Study the drawing (mm; zero at the part's minimum x, y, z) and answer. A direction names the side the tool comes from. Round coordinates to 2 decimals unless told otherwise and drop trailing zeros. Write each loop counter-clockwise with the first axis right and the second up, starting at its lowest first coordinate (ties: lowest second). Pieces come first, ordered by that corner, then holes.
(1) Each of these flat-tipped pins is pushed along its axis until it touches: pin 1 Ø1 at (x, y) = (1.5, 6.5) entering from -Z; pin 2 Ø0.7 at (x, y) = (3, 2) entering from +Z. Where does it stop, or does it pass through?
(2) Find the intervals of material crossed by probe 1 along Z at (x, y) = (2.35, 2.5); probe 2 along X at (y, z) = (3.75, 2.35); probe 3 along X at (y, z) = (22.75, 1.5), in increasing order.
(3) A cutting plane is placed at A-A, the plane y = 21.25. Give the vertices of the cut face in (x, z).
(4) For the marked faces 1 and 2, determine the directions among +Z, -Z, +X, -X, +Y, -Y from which every point of the face is accessible in a straight line to the end or side of a thin tool.
(5) A cutting plane is placed at B-B, the plane y = 3. Give the vertices of the cut face in (x, z), and give its area (3 significant figures).
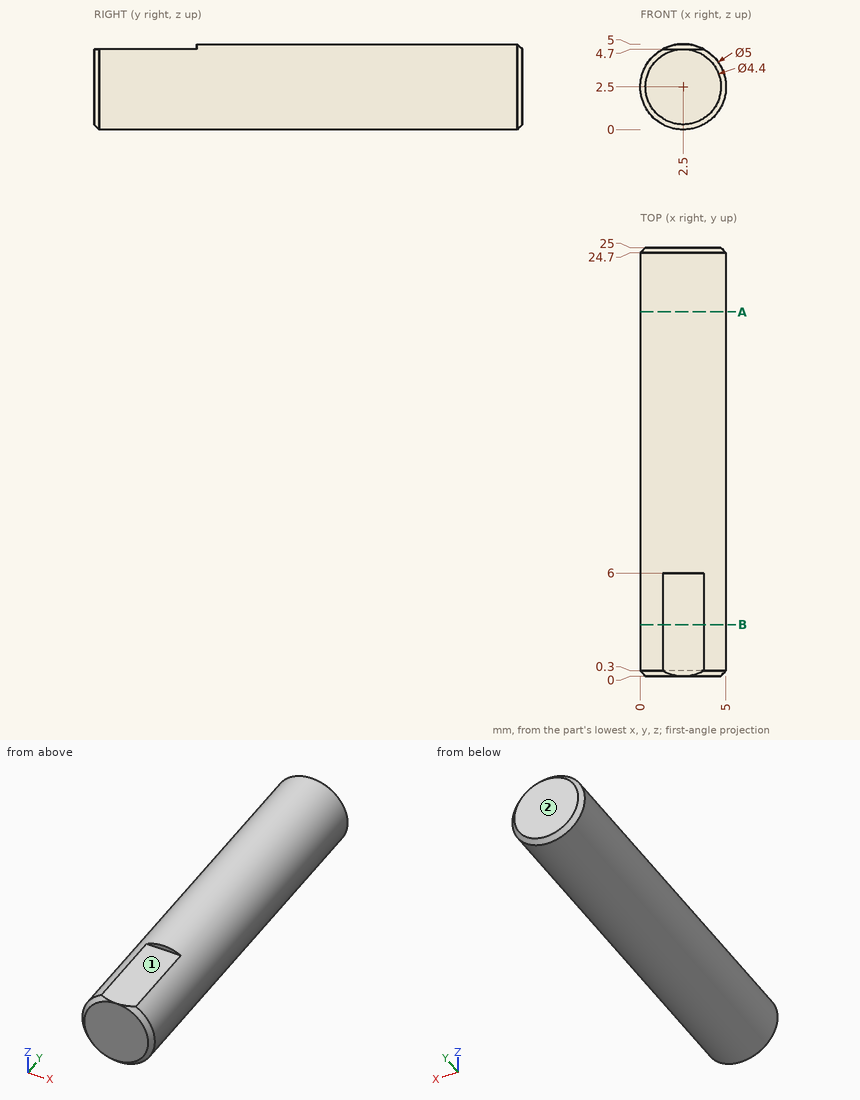
Solutions:
1. pin 1: stops at z = 0.05
1. pin 2: stops at z = 4.7
2. probe 1: z = 0 to 4.7
2. probe 2: x = 0 to 5
2. probe 3: x = 0.21 to 4.79
3. outline: circle Ø5 at (2.5, 2.5)
4. face 1: +Z, +X, -X, -Y
4. face 2: +Z, -Z, +X, -X, +Y
5. outline: (1.31, 4.7) arc R2.5 ccw (long way) to (3.69, 4.7) - close
5. area: 19.2 mm2
